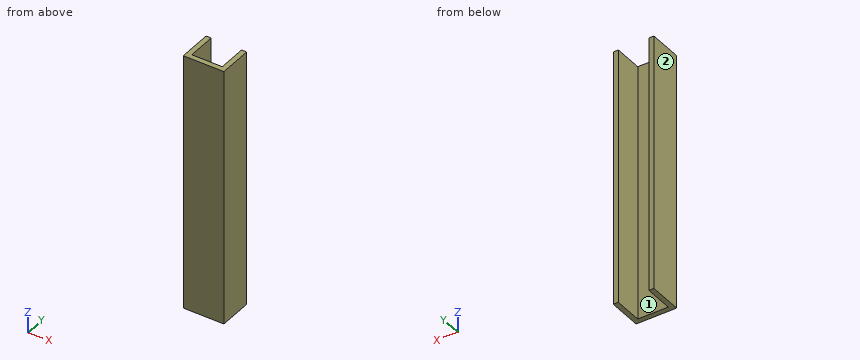
```python
from build123d import *

# Parameters (mm, degrees)
EXTRUDE_1_DEPTH     = 45
SKETCH_2_W          = 15
SKETCH_2_H          = 12
CUT_EXTRUDE_1_DEPTH = 10


with BuildPart() as part:
    # 草图1 → 凸台-拉伸1 (new, symmetric)
    with BuildSketch(Plane.XY):
        Polygon((-6, -5), (6, -5), (6, 5), (4.5, 5), (4.5, -3.5), (-4.5, -3.5), (-4.5, 5), (-6, 5), align=None)
    extrude(amount=EXTRUDE_1_DEPTH, both=True)

    # 草图2 → 切除-拉伸1 (cut, symmetric)
    with BuildSketch(Plane(origin=(0, 0, 0), x_dir=(0, 0, -1), z_dir=(1, 0, 0))):
        with Locations((-38.5, 0)):
            Rectangle(SKETCH_2_W, SKETCH_2_H)
    extrude(amount=CUT_EXTRUDE_1_DEPTH, both=True, mode=Mode.SUBTRACT)


solid = part.part
```
CAD build for the part. Positions are in the model's coordinates, mm. Face numbers are marked on the shaded views. A direction names the side the tool comes from. Coordinates: 2 decimals unless noted, no trailing zeros. Order: outer loops, then holes, each group sorted by start corner. A loop starts at its lowest first (then second) coordinate and runs counter-clockwise, first axis right, second up.
(1) Saw through at C-C, the plane x = 3.5. Write the cut outline in (y, z), and give its area (3 significant figures).
Solution:
outline: (-5, -45) - (-3.5, -45) - (-3.5, 31) - (-5, 31) - close
area: 114 mm2
(2) Which spindle directions (+Z, -Z, +X, -X, +Y, -Y) get a long thin tool onto all of the face, cutting with end or side? Do the marked faces 1 and 2. Say none if no direction does.
Solution:
face 1: +Z, -Z, +Y
face 2: +Z, -Z, -X, +Y, -Y
(3) Saw through at A-A, the plane y = 0.5. Write the cut outline in (x, z), and give its area (3 significant figures).
Solution:
outline: (-6, -45) - (-4.5, -45) - (-4.5, 31) - (-6, 31) - close; (4.5, -45) - (6, -45) - (6, 31) - (4.5, 31) - close
area: 228 mm2
(4) Drill centre lines: L1, parallel to X at y = 4.75, z = -19.5; L2, parallel to Y at x = -2.5, z = -36.5. Where is each one in solid material? Low to high.
Solution:
L1: x = -6 to -4.5, 4.5 to 6
L2: y = -5 to -3.5
(5) Saw through at B-B, the plane z = -17. Write the cut outline in (x, y), and give its area (3 significant figures).
Solution:
outline: (-6, -5) - (6, -5) - (6, 5) - (4.5, 5) - (4.5, -3.5) - (-4.5, -3.5) - (-4.5, 5) - (-6, 5) - close
area: 43.5 mm2
